```python
from build123d import *

# Parameters (mm, degrees)
SKETCH_2_4_R        = 2.6035
SKETCH_2_4_W        = 96.195388
SKETCH_2_4_H        = 6.300216
BOSS_EXTRUDE2_DEPTH = 1.7
SKETCH_2_4_2_W      = 96.195388
SKETCH_2_4_2_H      = 6.300216
BOSS_EXTRUDE3_DEPTH = 10.5
SKETCH4_W           = 3.597592
SKETCH4_H           = 6.300216
SKETCH4_W_2         = 3.597836
CUT_EXTRUDE1_DEPTH  = 8.8
SKETCH3_W           = 71.2
SKETCH3_H           = 2.100216
SKETCH3_W_2         = 12
SKETCH3_H_2         = 2.1
CUT_EXTRUDE2_DEPTH  = 8
MOVE_FACE1_BY       = 0.3
MOVE_FACE1_2_BY     = 0.3
MOVE_FACE1_3_BY     = 0.3


with BuildPart() as part:
    # Sketch 2_4 → Boss-Extrude2 (new body)
    # profile 1 of 2: a face of its own
    with BuildSketch(Plane(origin=(0, 0, 0), x_dir=(1, 0, 0), z_dir=(0, 1, 0))):
        with BuildLine():
            Line((134.543292, 0), (0.999998, 0))
            ThreePointArc((0.999998, 0), (0.292896914, 0.292896914), (0, 0.999998))
            Line((0, 0.999998), (0, 15.80007))
            ThreePointArc((0, 15.80007), (0.292907414, 16.507160586), (0.999998, 16.800068))
            Line((0.999998, 16.800068), (28.450032, 16.800068))
            ThreePointArc((28.450032, 16.800068), (29.157130586, 16.507168586), (29.45003, 15.80007))
            Line((29.45003, 15.80007), (29.45003, 14.800072))
            ThreePointArc((29.45003, 14.800072), (29.742916414, 14.092960414), (30.450028, 13.800074))
            Line((30.450028, 13.800074), (110.949994, 13.800074))
            ThreePointArc((110.949994, 13.800074), (111.657114586, 14.092951414), (111.949992, 14.800072))
            Line((111.949992, 14.800072), (111.949992, 15.80007))
            ThreePointArc((111.949992, 15.80007), (112.242900414, 16.507159586), (112.94999, 16.800068))
            Line((112.94999, 16.800068), (145.999962, 16.800068))
            ThreePointArc((145.999962, 16.800068), (146.707067586, 16.507175586), (146.99996, 15.80007))
            Line((146.99996, 15.80007), (146.99996, 1.49987))
            ThreePointArc((146.99996, 1.49987), (146.707065586, 0.792766414), (145.999962, 0.499872))
            Line((145.999962, 0.499872), (135.866124, 0.499872))
            ThreePointArc((135.866124, 0.499872), (135.512587346, 0.435316415), (135.204708, 0.249936))
            ThreePointArc((135.204708, 0.249936), (134.896826655, 0.064560877), (134.543292, 0))
        make_face()
        with Locations(Location((140.999972, 10.500106, 0), (0, 0, 270))):
            Circle(SKETCH_2_4_R, mode=Mode.SUBTRACT)
        with Locations(Location((5.999988, 5.999988, 0), (0, 0, 270))):
            Circle(SKETCH_2_4_R, mode=Mode.SUBTRACT)
        with Locations((70.999858, 3.899916)):
            Rectangle(SKETCH_2_4_W, SKETCH_2_4_H, mode=Mode.SUBTRACT)
    # profile 2 of 2: a face of its own
    with BuildSketch(Plane(origin=(0, 0, 0), x_dir=(1, 0, 0), z_dir=(0, 1, 0))):
        with Locations((70.999858, 3.899916)):
            Rectangle(SKETCH_2_4_W, SKETCH_2_4_H)
    extrude(amount=BOSS_EXTRUDE2_DEPTH)

    # Sketch 2_4 2 → Boss-Extrude3 (add)
    with BuildSketch(Plane(origin=(0, 0, 0), x_dir=(1, 0, 0), z_dir=(0, 1, 0))):
        with Locations((70.999858, 3.899916)):
            Rectangle(SKETCH_2_4_2_W, SKETCH_2_4_2_H)
    extrude(amount=BOSS_EXTRUDE3_DEPTH)

    # Sketch4 → Cut-Extrude1 (cut)
    with BuildSketch(Plane(origin=(0, 10.5, 0), x_dir=(1, 0, 0), z_dir=(0, 1, 0))):
        with Locations((117.298756, 3.899916)):
            Rectangle(SKETCH4_W, SKETCH4_H)
        with Locations((24.701082, 3.899916)):
            Rectangle(SKETCH4_W_2, SKETCH4_H)
    extrude(amount=-CUT_EXTRUDE1_DEPTH, mode=Mode.SUBTRACT)

    # Sketch3 → Cut-Extrude2 (cut)
    with BuildSketch(Plane(origin=(0, 10.5, 0), x_dir=(1, 0, 0), z_dir=(0, 1, 0))):
        with Locations((63.5, 3.899916)):
            Rectangle(SKETCH3_W, SKETCH3_H)
        with Locations((106.9, 3.899808)):
            Rectangle(SKETCH3_W_2, SKETCH3_H_2)
    extrude(amount=-CUT_EXTRUDE2_DEPTH, mode=Mode.SUBTRACT)

    # Move Face1: a face moved outward by 0.3
    extrude(part.faces().sort_by_distance((63.5, 6.5, -4.950024))[0], amount=MOVE_FACE1_BY, dir=(0, 0, 1))

    # Move Face1 2: a face moved inward by 0.3
    extrude(part.faces().sort_by_distance((70.99998, 6.1, -7.050024))[0], amount=MOVE_FACE1_2_BY, dir=(0, 0, 1), mode=Mode.SUBTRACT)

    # Move Face1 3: a face moved outward by 0.3
    extrude(part.faces().sort_by_distance((106.9, 6.5, -4.949808))[0], amount=MOVE_FACE1_3_BY, dir=(0, 0, 1))


solid = part.part
```
Input: part model. Units: mm. Frame: model coordinates. A direction names the side the tool comes from. Coordinates: 2 decimals unless noted, no trailing zeros. Loops run counter-clockwise (first coordinate to the right, second up) from the corner with the lowest first, then second, coordinate; pieces in that order, holes last. Notation, with made-up numbers: M 29,-27.75 L 35,-27.75 A19 ccw 35,-19.75 Z; hole C 59,52 d3. An arc over 180 degrees is marked long. Answer in a Markdown table with one row per item.
1. Reachability of faces 5 (the flat face through (70, 6, -6.75)), 6 (the flat face through (63, 7, -4.65)), 7 (the flat face through (72, 0, -9)), 8 (the flat face through (115.5, 6, -4)) from +Z, -Z, +X, -X, +Y, -Y: full face, straight path, thin tool, end or side. Return the list, or none.
Response:
| item | result |
|---|---|
| face 5 | -Z, +X, -X, +Y |
| face 6 | +Y |
| face 7 | +Z, -Z, +X, -X, -Y |
| face 8 | +Z, -Z, +X, +Y |
2. Draft query along Z for faces 1 (the flat face through (26.5, 6, -4)), 2 (the flat face through (63, 7, -2.85)), 3 (the flat face through (70, 6, -0.75)), 4 (the flat face through (107, 7, -4.65)). Return one class per face: pulls with the +Z half, pulls with the -Z half, needs draft (parallel to the pull), parting line crosses it, or undercut.
Response:
| item | result |
|---|---|
| face 1 | needs draft |
| face 2 | undercut |
| face 3 | pulls with the +Z half |
| face 4 | undercut |
3. Section D-D, the plane x = 12.5. Output: boundary loops of the cut face in (y, z).
Response:
| item | result |
|---|---|
| outline | M 0,-16.8 L 1.7,-16.8 L 1.7,0 L 0,0 Z |
4. First-contact query: pin 1 (2 mm diameter, centred on x = 40.5, z = -10.5, fed in from +Y); pin 2 (4 mm diameter, centred on x = 81, y = 7, fed in from -Z); pin 3 (2.5 mm diameter, centred on x = 78.5, y = 5.5, fed in from +Z); pin 4 (4.5 mm diameter, centred on x = 141, z = -10.5, fed in from +Y). Flat tips, straight axial feed; report the tip coordinate or a pass-through.
Response:
| item | result |
|---|---|
| pin 1 | stops at y = 1.7 |
| pin 2 | stops at z = -6.75 |
| pin 3 | stops at z = -0.75 |
| pin 4 | passes through |
5. Section A-A, the plane y = 6. Output: boundary loops of the cut face in (x, z).
Response:
| item | result |
|---|---|
| outline | M 26.5,-6.75 L 115.5,-6.75 L 115.5,-0.75 L 26.5,-0.75 Z; hole M 27.9,-4.65 L 99.1,-4.65 L 99.1,-2.85 L 27.9,-2.85 Z; hole M 100.9,-4.65 L 112.9,-4.65 L 112.9,-2.85 L 100.9,-2.85 Z |
6. Material intervals for line 1 (Z direction, x = 44, y = 6.5); line 2 (X direction, y = 4.5, z = -3.25); line 3 (X direction, y = 6, z = -1), sorted ascending.
Response:
| item | result |
|---|---|
| line 1 | z = -6.75 to -4.65, -2.85 to -0.75 |
| line 2 | x = 26.5 to 27.9, 99.1 to 100.9, 112.9 to 115.5 |
| line 3 | x = 26.5 to 115.5 |
7. Section B-B, the plane x = 103.5. Output: boundary loops of the cut face in (y, z).
Response:
| item | result |
|---|---|
| outline | M 0,-13.8 L 1.7,-13.8 L 1.7,-6.75 L 10.5,-6.75 L 10.5,-4.65 L 2.5,-4.65 L 2.5,-2.85 L 10.5,-2.85 L 10.5,-0.75 L 1.7,-0.75 L 1.7,0 L 0,0 Z |
